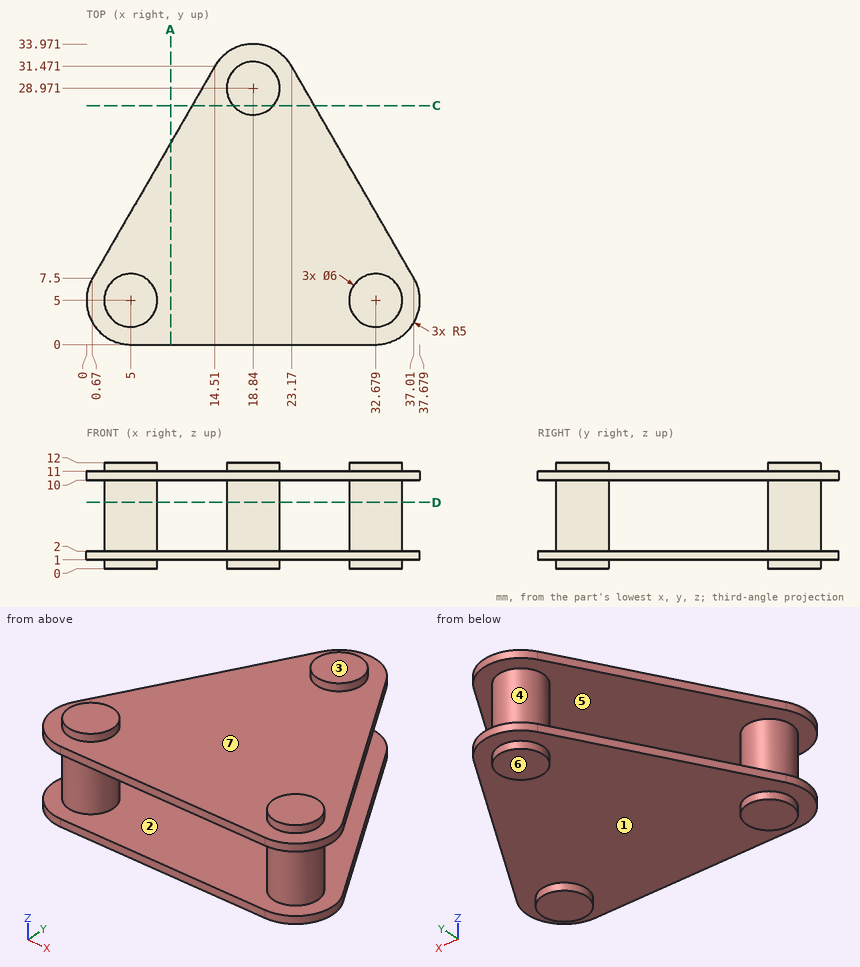
Verification items for this drawing (mm, ordinates from the low corner). A direction names the side the tool comes from. Coordinates: 2 decimals unless noted, no trailing zeros. Order: outer loops, then holes, each group sorted by start corner. A loop starts at its lowest first (then second) coordinate and runs counter-clockwise, first axis right, second up. Notation, with made-up numbers: (68.25, -11) -> (93.25, -11) arc R22 cw to (93.25, 19) -> close; hole circle Ø1 at (53, 1). An arc over 180 degrees is marked (long way). Put each result on its own line as item: value. Start each with the question number.
1. Cross-section at D-D, the plane z = 7.5. Record the boundary of the cut face in (x, y).
2. Mould release check, pull along X, two halves, no side actions. Record for the marked faces 4, 5, 6 and 7: released by +X, released by -X, zero draft, split by the parting line, or undercut.
3. Access from +Z, -Z, +X, -X, +Y, -Y to the whole of each face (thin tool, end or side, straight path). Record for the marked faces 1, 2 and 3.
4. Cross-section at C-C, the plane y = 27. Record the boundary of the cut face in (x, z).
5. Go/stop test with flat-tipped pins: pin 1 Ø2 at (x, y) = (20.5, 13) entering from +Z; pin 2 Ø10 at (x, y) = (20, 12.5) entering from -Z; pin 3 Ø1.5 at (y, z) = (20, 10) entering from +X (1 decimal). Record where each tip stops, or that it passes through.
6. Material ranges on L1, parallel to Z at x = 8, y = 9.5; L2, parallel to Y at x = 4, z = 9.75; L3, parallel to X at y = 30.5, z = 9.5, recorded low to high. Write a range as [from, to].
7. Cross-section at A-A, the plane x = 9.5. Record the boundary of the cut face in (y, z) (1 decimal).
Computed:
1. outline: circle Ø6 at (5, 5); circle Ø6 at (18.84, 28.97); circle Ø6 at (32.68, 5)
2. face 4: split by the parting line
2. face 5: undercut
2. face 6: zero draft
2. face 7: undercut
3. face 1: -Z
3. face 2: none
3. face 3: +Z, +X, -X, +Y, -Y
4. outline: (11.93, 1) -> (16.58, 1) -> (16.58, 0) -> (21.1, 0) -> (21.1, 1) -> (25.75, 1) -> (25.75, 2) -> (21.1, 2) -> (21.1, 10) -> (25.75, 10) -> (25.75, 11) -> (21.1, 11) -> (21.1, 12) -> (16.58, 12) -> (16.58, 11) -> (11.93, 11) -> (11.93, 10) -> (16.58, 10) -> (16.58, 2) -> (11.93, 2) -> close
5. pin 1: z = 11
5. pin 2: z = 1
5. pin 3: x = 30.2
6. L1: [1, 2], [10, 11]
6. L2: [2.17, 7.83]
6. L3: [16.26, 21.42]
7. outline: (0, 1) -> (22.8, 1) -> (22.8, 2) -> (0, 2) -> close; (0, 10) -> (22.8, 10) -> (22.8, 11) -> (0, 11) -> close
